Part model, mm, in its own coordinate system. Face numbers are marked on the shaded views. A direction names the side the tool comes from. Give positions to 0.01 mm unless a question says otherwise; leave off trailing zeros. Write each loop counter-clockwise with the first axis right and the second up, starting at its lowest first coordinate (ties: lowest second). Pieces come first, ordered by that corner, then holes. Notation, with made-up numbers: (-4.5, 30.25) - (35.5, 30.25) arc R21 cw to (35.5, 67.25) - close; hole circle Ø5 at (-16, 4.5). An arc over 180 degrees is marked (long way). Answer as a JSON object with one key per item and string values. Group by question number.
```python
from build123d import *

# Parameters (mm, degrees)
EXTRUDE_1_DEPTH     = 120
SKETCH_2_R          = 8.6
CUT_EXTRUDE_1_DEPTH = 142.449637681


with BuildPart() as part:
    # 草图1 → 凸台-拉伸1 (new body)
    with BuildSketch(Plane(origin=(0, 0, 0), x_dir=(1, 0, 0), z_dir=(0, 1, 0))):
        Polygon((62, 11), (10, 11), (10, -11), (62, -11), (62, -21), (0, -21), (0, 21), (62, 21), align=None)
    extrude(amount=EXTRUDE_1_DEPTH)

    # 草图2 → 切除-拉伸1 (cut, through all)
    with BuildSketch(Plane.XY.offset(21)):
        with Locations((42, 100)):
            Circle(SKETCH_2_R)
        with Locations((42, 20)):
            Circle(SKETCH_2_R)
    extrude(amount=-CUT_EXTRUDE_1_DEPTH, mode=Mode.SUBTRACT)


solid = part.part
```
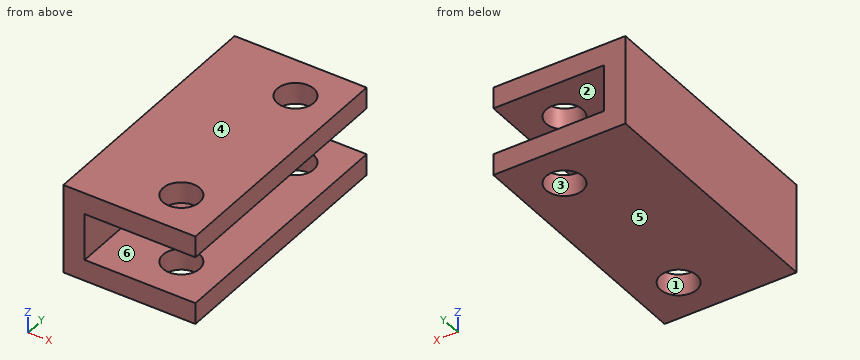
1) Saw through at C-C (y = 100). List the corners of the cut face in (x, z), and give its area (3 significant figures).
2) Drill centre lines: line 1 along Y through (x, z) = (42, 17.25); line 2 along Z through (x, y) = (18, 112.5); line 3 along X through (y, z) = (85, 3). Where is each one in solid material? Low to high. Write a range as from..to.
3) Saw through at B-B (z = -13). List the corners of the cut face in (x, y), and give its area (3 significant figures).
4) Two-plate mould, pull along Z, no slides. Class the marked faces 3, 4, 5 and 6: +Z half, -Z half, draft (parallel to the pull), parting line (faces both ways), or undercut.
5) Which spindle directions (+Z, -Z, +X, -X, +Y, -Y) get a long thin tool onto all of the face, cutting with end or side? Do the marked faces 1 and 2. Say none if no direction does.
6) Drop flat-ended pins along their axis: P1, Ø14, axis at x = 42, y = 100, coming from the +Z side; P2, Ø6.5, axis at y = 75.5, z = -1, coming from the +X side. Give the stop position or say it passes through.
7) Saw through at A-A (x = 42). List the corners of the cut face in (y, z).
8) Saw through at D-D (x = 14). List the corners of the cut face in (y, z).
Checks:
{
 "1": {"outline": "(0, -21) - (33.4, -21) - (33.4, -11) - (10, -11) - (10, 11) - (33.4, 11) - (33.4, 21) - (0, 21) - close; (50.6, -21) - (62, -21) - (62, -11) - (50.6, -11) - close; (50.6, 11) - (62, 11) - (62, 21) - (50.6, 21) - close", "area": "1,120 mm2"},
 "2": {"line 1": "0..11.4, 28.6..91.4, 108.6..120", "line 2": "-21..-11, 11..21", "line 3": "0..10"},
 "3": {"outline": "(0, 0) - (62, 0) - (62, 120) - (0, 120) - close; hole circle Ø17.2 at (42, 20); hole circle Ø17.2 at (42, 100)", "area": "6,980 mm2"},
 "4": {"face 3": "draft", "face 4": "+Z half", "face 5": "-Z half", "face 6": "undercut"},
 "5": {"face 1": "+Z, -Z", "face 2": "+X, +Y, -Y"},
 "6": {"P1": "through", "P2": "x = 10"},
 "7": {"outline": "(0, -21) - (11.4, -21) - (11.4, -11) - (0, -11) - close; (0, 11) - (11.4, 11) - (11.4, 21) - (0, 21) - close; (28.6, -21) - (91.4, -21) - (91.4, -11) - (28.6, -11) - close; (28.6, 11) - (91.4, 11) - (91.4, 21) - (28.6, 21) - close; (108.6, -21) - (120, -21) - (120, -11) - (108.6, -11) - close; (108.6, 11) - (120, 11) - (120, 21) - (108.6, 21) - close"},
 "8": {"outline": "(0, -21) - (120, -21) - (120, -11) - (0, -11) - close; (0, 11) - (120, 11) - (120, 21) - (0, 21) - close"}
}
